from build123d import *

# Parameters (mm, degrees)
EXTRUDE1_DEPTH = 10


with BuildPart() as part:
    # Sketch1 → Revolve1 (revolve)
    with BuildSketch(Plane.XY, mode=Mode.PRIVATE) as revolve1_sk:
        Polygon((0, 0), (50, 0), (50, 10), (45, 10), (13.404628949, 15), (13.404628949, 20), (10, 20), (10, 200), (0, 200), align=None)
    revolve(revolve1_sk.sketch.rotate(Axis((0, 0, 0), (0, 1, 0)), 90), axis=Axis((0, 0, 0), (0, 1, 0)))

    # Sketch2 → Extrude1 (add)
    with BuildSketch(Plane.XZ.offset(-110)):
        Polygon((0, 17.320508076), (-15, 8.660254038), (-15, -8.660254038), (0, -17.320508076), (15, -8.660254038), (15, 8.660254038), align=None)
    extrude(amount=EXTRUDE1_DEPTH)


solid = part.part
Geometry check sheet. Reference: the model listing, model coordinates, mm. A direction names the side the tool comes from. Round coordinates to 2 decimals unless told otherwise and drop trailing zeros. Loops run counter-clockwise (first coordinate to the right, second up) from the corner with the lowest first, then second, coordinate; pieces in that order, holes last. Notation, with made-up numbers: (-22.75, 63) - (11.25, 63) arc R15 ccw to (11.25, 80) - close; hole circle Ø9 at (76, 74). An arc over 180 degrees is marked (long way). One line per question, with ' | ' between items. Start each with the question number.
1. Cross-section at B-B on y = 165. Record the cut outline in (x, z).
2. Scan lines: line 1 (Z direction, x = 5, y = 139); line 2 (Y direction, x = -18.5, z = -14); line 3 (X direction, y = 109, z = 2.5). Record each from-to range of solid material in increasing order. Write a range as [from, to].
3. Tool access check on faces 1 (the face through (-6.9, 110, -7.5)), 2 (the face through (9, 20, 5)), 3 (the face through (-7.605, 105.07, -12.93)). Record the directions out of +Z, -Z, +X, -X, +Y, -Y that give a thin tool (end or side, any length) a straight path to the whole face; none if there is none.
4. Depth check by flat-ended pin: pin 1 (9 mm diameter, centred on x = 5.5, z = -7.5, fed in from -Y); pin 2 (2 mm diameter, centred on y = 50, z = -8, fed in from -X); pin 3 (8 mm diameter, centred on y = 107, z = 3.5, fed in from +X); pin 4 (8 mm diameter, centred on x = -14.5, z = 10, fed in from +Y). Enter the tip coordinate at first touch or a pass-through.
5. Cross-section at A-A on z = 0. Record the cut outline in (x, y).
Taken from the geometry:
1) outline: circle Ø20 at (0, 0)
2) line 1: [-8.66, 8.66] | line 2: [0, 13.45] | line 3: [-15, 15]
3) face 1: +Y | face 2: none | face 3: -Z, -X, +Y
4) pin 1: y = 0 | pin 2: x = -7.14 | pin 3: x = 15 | pin 4: y = 110
5) outline: (-50, 0) - (50, 0) - (50, 10) - (45, 10) - (13.4, 15) - (13.4, 20) - (10, 20) - (10, 100) - (15, 100) - (15, 110) - (10, 110) - (10, 200) - (-10, 200) - (-10, 110) - (-15, 110) - (-15, 100) - (-10, 100) - (-10, 20) - (-13.4, 20) - (-13.4, 15) - (-45, 10) - (-50, 10) - close
